Part model, mm, in its own coordinate system. Face numbers are marked on the shaded views. A direction names the side the tool comes from. Coordinates: 2 decimals unless noted, no trailing zeros. Write each loop counter-clockwise with the first axis right and the second up, starting at its lowest first coordinate (ties: lowest second). Pieces come first, ordered by that corner, then holes. Notation, with made-up numbers: (-24.5, 18.25) - (7.5, 18.25) arc R29 ccw to (7.5, 42.25) - close; hole circle Ø6 at (25.25, 53.25). An arc over 180 degrees is marked (long way). Write each question's results on one line, items separated by ' | '.
from build123d import *

# Parameters (mm, degrees)
BASE_DISC_SKETCH_R     = 31
BASE_DISC_62_DEPTH     = 8
SQUARE_CUT_SKETCH_R    = 5
SQUARE_CUT_10X10_DEPTH = 8
JAWS_DEPTH             = 20
JAW_NOTCH_1_DEPTH      = 10
JAW_NOTCH_2_DEPTH      = 10
JAW_NOTCH_3_DEPTH      = 10
JAW_NOTCH_4_DEPTH      = 10
JAW_NOTCH_5_DEPTH      = 10
JAW_NOTCH_6_DEPTH      = 10
JAW_HOLE_1_SKETCH_R    = 3
JAW_HOLE_1_6_DEPTH     = 10
JAW_HOLE_2_SKETCH_R    = 3
JAW_HOLE_2_6_DEPTH     = 10
JAW_HOLE_3_SKETCH_R    = 3
JAW_HOLE_3_6_DEPTH     = 10
JAW_START              = -10
JAW_HOLE_4_SKETCH_R    = 3
JAW_HOLE_4_6_DEPTH     = 10
JAW_HOLE_5_SKETCH_R    = 3
JAW_HOLE_5_6_DEPTH     = 10
JAW_HOLE_6_SKETCH_R    = 3
JAW_HOLE_6_6_DEPTH     = 10
HOLE_15_SKETCH_R       = 7.5
HOLE_15_DEPTH          = 10


with BuildPart() as part:
    # Base Disc Sketch → Base Disc Ø62 (new body)
    with BuildSketch(Plane.XY):
        Circle(BASE_DISC_SKETCH_R)
    extrude(amount=BASE_DISC_62_DEPTH)

    # Square Cut Sketch → Square Cut 10x10 (cut)
    with BuildSketch(Plane.XY.offset(8)):
        with Locations((-17.67766953, 17.67766953)):
            Circle(SQUARE_CUT_SKETCH_R)
        with Locations((24.148145657, 6.470476128)):
            Circle(SQUARE_CUT_SKETCH_R)
        with Locations((-6.470476128, -24.148145657)):
            Circle(SQUARE_CUT_SKETCH_R)
    extrude(amount=-SQUARE_CUT_10X10_DEPTH, mode=Mode.SUBTRACT)

    # Jaws Sketch → Jaws (add)
    with BuildSketch(Plane.XY.offset(8)):
        with BuildLine():
            Line((-30.109514993, -7.376795165), (-9.961946981, -0.871557427))
            ThreePointArc((-9.961946981, -0.871557427), (-9.990482216, 0.436193874), (-9.84807753, 1.736481777))
            ThreePointArc((-9.84807753, 1.736481777), (-8.191520443, 5.735764364), (-5, 8.660254038))
            Line((-5, 8.660254038), (-5, 10))
            Line((-5, 10), (-5, 30.594117082))
            ThreePointArc((-5, 30.594117082), (-7.526051267, 30.072554802), (-10, 29.342801502))
            Line((-10, 29.342801502), (-10, 11.649864154))
            ThreePointArc((-10, 11.649864154), (-11.915260032, 5.764545161), (-16.927395931, 2.133609416))
            Line((-16.927395931, 2.133609416), (-30.908458268, -2.38058973))
            ThreePointArc((-30.908458268, -2.38058973), (-30.611089207, -4.895019672), (-30.109514993, -7.376795165))
        make_face()
        with BuildLine():
            ThreePointArc((4.226182617, -9.06307787), (-1.305261922, -9.914448614), (-6.427876097, -7.660444431))
            Line((-6.427876097, -7.660444431), (-7.686825491, -8.118664537))
            Line((-7.686825491, -8.118664537), (-27.038965344, -15.162267413))
            ThreePointArc((-27.038965344, -15.162267413), (-25.684896703, -17.357594343), (-24.153012612, -19.432755383))
            Line((-24.153012612, -19.432755383), (-6.276119738, -12.926098496))
            ThreePointArc((-6.276119738, -12.926098496), (-1.550656383, -12.40857609), (2.879846058, -14.131504261))
            Line((2.879846058, -14.131504261), (18.365137045, -24.974421741))
            ThreePointArc((18.365137045, -24.974421741), (20.347505117, -23.387582934), (22.193351369, -21.64382487))
            Line((22.193351369, -21.64382487), (5.323638261, -9.831524585))
            Line((5.323638261, -9.831524585), (4.226182617, -9.06307787))
        make_face()
        with BuildLine():
            ThreePointArc((10, 29.342801502), (7.526051267, 30.072554802), (5, 30.594117082))
            Line((5, 30.594117082), (5, 10))
            Line((5, 10), (5, 8.660254038))
            ThreePointArc((5, 8.660254038), (8.870108332, 4.617486132), (9.961946981, -0.871557427))
            Line((9.961946981, -0.871557427), (11.059402625, -1.640004142))
            Line((11.059402625, -1.640004142), (27.929115732, -13.452304428))
            ThreePointArc((27.929115732, -13.452304428), (28.950760409, -11.083928535), (29.771980199, -8.638819075))
            Line((29.771980199, -8.638819075), (14.264235636, 2.219820568))
            ThreePointArc((14.264235636, 2.219820568), (11.129891668, 5.793854879), (10, 10.411341011))
            Line((10, 10.411341011), (10, 29.342801502))
        make_face()
    extrude(amount=JAWS_DEPTH)

    # Jaw Notch 1 Sketch → Jaw Notch 1 (cut)
    with BuildSketch(Plane.ZY.offset(-5)):
        Polygon((28, 30.594117082), (28, 27.594117082), (24.316442961, 30.594117082), align=None)
    extrude(amount=-JAW_NOTCH_1_DEPTH, mode=Mode.SUBTRACT)

    # Jaw Notch 2 Sketch → Jaw Notch 2 (cut)
    with BuildSketch(Plane(origin=(-5, 0, 0), x_dir=(0, 0, -1), z_dir=(1, 0, 0))):
        Polygon((-28, 30.594117082), (-24.316442961, 30.594117082), (-28, 27.594117082), align=None)
    extrude(amount=-JAW_NOTCH_2_DEPTH, mode=Mode.SUBTRACT)

    # Jaw Notch 3 Sketch → Jaw Notch 3 (cut)
    with BuildSketch(Plane(origin=(2.867882182, 4.095760221, 0), x_dir=(0.8191520442889944, -0.5735764363510426, 0), z_dir=(-0.5735764363510426, -0.8191520442889944, 0))):
        Polygon((30.594117082, 28), (30.594117082, 25), (27.594117082, 28), align=None)
    extrude(amount=-JAW_NOTCH_3_DEPTH, mode=Mode.SUBTRACT)

    # Jaw Notch 4 Sketch → Jaw Notch 4 (cut)
    with BuildSketch(Plane(origin=(-2.867882182, -4.095760221, 0), x_dir=(0.8191520442889944, -0.5735764363510426, 0), z_dir=(0.5735764363510426, 0.8191520442889944, 0))):
        Polygon((27.594117082, -28), (30.594117082, -28), (30.594117082, -25), align=None)
    extrude(amount=-JAW_NOTCH_4_DEPTH, mode=Mode.SUBTRACT)

    # Jaw Notch 5 Sketch → Jaw Notch 5 (cut)
    with BuildSketch(Plane(origin=(-0.685656401, 2.123567121, 0), x_dir=(0.9516254737982698, 0.3072604068509618, 0), z_dir=(0.3072604068509618, -0.9516254737982698, 0))):
        Polygon((-30.919578554, 28), (-27.919578554, 28), (-30.919578554, 25), align=None)
    extrude(amount=-JAW_NOTCH_5_DEPTH, mode=Mode.SUBTRACT)

    # Jaw Notch 6 Sketch → Jaw Notch 6 (cut)
    with BuildSketch(Plane(origin=(1.710100717, -4.698463104, 0), x_dir=(0.9396926207859072, 0.34202014332567215, 0), z_dir=(-0.3420201433256721, 0.9396926207859071, 0))):
        Polygon((-27.635003822, -28), (-30.594117082, -25.550278158), (-30.594117082, -28), align=None)
    extrude(amount=-JAW_NOTCH_6_DEPTH, mode=Mode.SUBTRACT)

    # Jaw Hole 1 Sketch → Jaw Hole 1 Ø6 (cut)
    with BuildSketch(Plane(origin=(-0.685656401, 2.123567121, 0), x_dir=(0.9516254737982698, 0.3072604068509618, 0), z_dir=(0.3072604068509618, -0.9516254737982698, 0))):
        with Locations((-22.919578554, 21.853934113)):
            Circle(JAW_HOLE_1_SKETCH_R)
    extrude(amount=-JAW_HOLE_1_6_DEPTH, mode=Mode.SUBTRACT)

    # Jaw Hole 2 Sketch → Jaw Hole 2 Ø6 (cut)
    with BuildSketch(Plane(origin=(1.710100717, -4.698463104, 0), x_dir=(0.9396926207859072, 0.34202014332567215, 0), z_dir=(-0.3420201433256721, 0.9396926207859071, 0))):
        with Locations(Location((-22.638380403, -21.853934113, 0), (0, 0, 180))):
            Circle(JAW_HOLE_2_SKETCH_R)
    extrude(amount=-JAW_HOLE_2_6_DEPTH, mode=Mode.SUBTRACT)

    # Jaw Hole 3 Sketch → Jaw Hole 3 Ø6 (cut)
    with BuildSketch(Plane.ZY.offset(-5)):
        with Locations((22, 21.342801502)):
            Circle(JAW_HOLE_3_SKETCH_R)
    extrude(amount=-JAW_HOLE_3_6_DEPTH, mode=Mode.SUBTRACT)

    # Jaw Hole 4 Sketch → Jaw Hole 4 Ø6 (cut)
    with BuildSketch(Plane(origin=(-5, 0, 0), x_dir=(0, 0, -1), z_dir=(1, 0, 0)).offset(JAW_START)):
        with Locations(Location((-22, 21.342801502, 0), (0, 0, 180))):
            Circle(JAW_HOLE_4_SKETCH_R)
    extrude(amount=JAW_HOLE_4_6_DEPTH, mode=Mode.SUBTRACT)

    # Jaw Hole 5 Sketch → Jaw Hole 5 Ø6 (cut)
    with BuildSketch(Plane(origin=(2.867882182, 4.095760221, 0), x_dir=(0.8191520442889944, -0.5735764363510426, 0), z_dir=(-0.5735764363510426, -0.8191520442889944, 0))):
        with Locations((21.368579376, 22)):
            Circle(JAW_HOLE_5_SKETCH_R)
    extrude(amount=-JAW_HOLE_5_6_DEPTH, mode=Mode.SUBTRACT)

    # Jaw Hole 6 Sketch → Jaw Hole 6 Ø6 (cut)
    with BuildSketch(Plane(origin=(-2.867882182, -4.095760221, 0), x_dir=(0.8191520442889944, -0.5735764363510426, 0), z_dir=(0.5735764363510426, 0.8191520442889944, 0)).offset(JAW_START)):
        with Locations((21.368579376, -22)):
            Circle(JAW_HOLE_6_SKETCH_R)
    extrude(amount=JAW_HOLE_6_6_DEPTH, mode=Mode.SUBTRACT)

    # Hole Ø15 Sketch → Hole Ø15 (cut)
    with BuildSketch(Plane.XY.offset(8)):
        Circle(HOLE_15_SKETCH_R)
    extrude(amount=-HOLE_15_DEPTH, mode=Mode.SUBTRACT)


solid = part.part
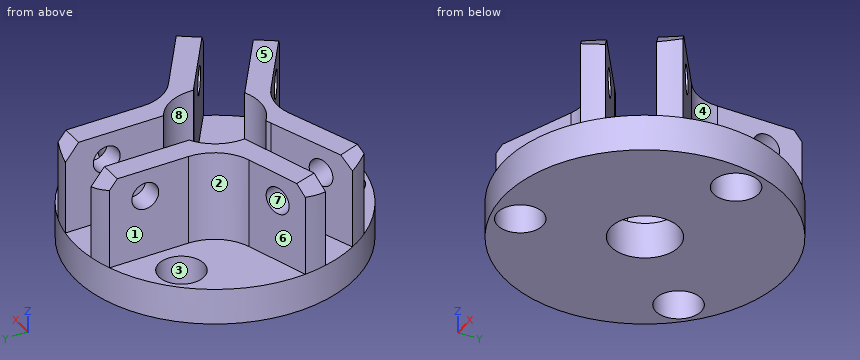
(1) Flat gauge pins, fed straight in: P1, Ø16, axis at y = 23, z = 23, coming from the -X side; P2, Ø12, axis at x = -8, z = 23.5, coming from the +Y side; P3, Ø4, axis at x = 5, y = 22, coming from the -Z side; P4, Ø8, axis at x = -9.5, z = 18.5, coming from the -Y side. Where does each tip first touch, or does it go through?
Return value:
P1: stops at x = -10 | P2: stops at y = 30.59 | P3: stops at z = 0 | P4: stops at y = -15.56
(2) Saw through at B-B on z = 12. Write the cut outline in (x, y).
Return value:
outline: (-30.91, -2.38) arc R31 ccw to (-30.11, -7.38) - (-9.96, -0.87) arc R10 cw to (-5, 8.66) - (-5, 30.59) arc R31 ccw to (-10, 29.34) - (-10, 11.65) arc R10 cw to (-16.93, 2.13) - close; (-27.04, -15.16) arc R31 ccw to (-24.15, -19.43) - (-6.28, -12.93) arc R10 cw to (2.88, -14.13) - (18.37, -24.97) arc R31 ccw to (22.19, -21.64) - (4.23, -9.06) arc R10 cw to (-6.43, -7.66) - close; (5, 8.66) arc R10 cw to (9.96, -0.87) - (27.93, -13.45) arc R31 ccw to (29.77, -8.64) - (14.26, 2.22) arc R10 cw to (10, 10.41) - (10, 29.34) arc R31 ccw to (5, 30.59) - close
(3) Wall check: line 1 (X direction, y = 24.5, z = 8.5); line 2 (X direction, y = 0.5, z = 2.25); line 3 (Y direction, x = -5.95, z = 22). Give the ranges that are in metal, low to high. Write a range as from..to.
Return value:
line 1: x = -10..-5, 5..10 | line 2: x = -31..-7.48, 7.48..31 | line 3: y = -12.81..-8.04, 8.04..18.34, 24.34..30.42
(4) Saw through at A-A on y = 13.5. Write the cut outline in (x, z), then the cut area to 3 significant figures.
Return value:
outline: (-27.91, 0) - (-20.42, 0) - (-20.42, 8) - (-27.91, 8) - close; (-14.93, 0) - (27.91, 0) - (27.91, 8) - (10, 8) - (10, 28) - (5, 28) - (5, 8) - (-5, 8) - (-5, 28) - (-10, 28) - (-10, 8) - (-14.93, 8) - close | area: 603 mm^2
(5) 3-axis set-ups, long thin cutter, end or side, ignore diameter. For the marked faces 4, 5, 6, 7 and 8: which of +Z, -Z, +X, -X, +Y, -Y reach the whole face in a straight line?
Return value:
face 4: +Z, +X, +Y | face 5: +Z, +X, -X, +Y, -Y | face 6: +Z, -X, +Y | face 7: none | face 8: +Z
(6) Two-plate mould, pull along Y, no slides. Class the marked faces 1, 2 and 3: released by +Y, released by -Y, zero draft, split by the parting line, or undercut.
Return value:
face 1: zero draft | face 2: released by +Y | face 3: undercut
(7) Saw through at D-D on y = -26. Write the cut outline in (x, z), then the cut area to 3 significant figures.
Return value:
outline: (-16.88, 0) - (-11.11, 0) - (-11.11, 8) - (-16.88, 8) - close; (-1.83, 0) - (16.88, 0) - (16.88, 8) - (-1.83, 8) - close | area: 196 mm^2
(8) Saw through at C-C on x = 0. Write the cut outline in (y, z), then the cut area to 3 significant figures.
Return value:
outline: (-31, 0) - (-7.5, 0) - (-7.5, 8) - (-10, 8) - (-10, 28) - (-12.74, 28) - (-12.74, 8) - (-31, 8) - close; (7.5, 0) - (31, 0) - (31, 8) - (7.5, 8) - close | area: 431 mm^2
